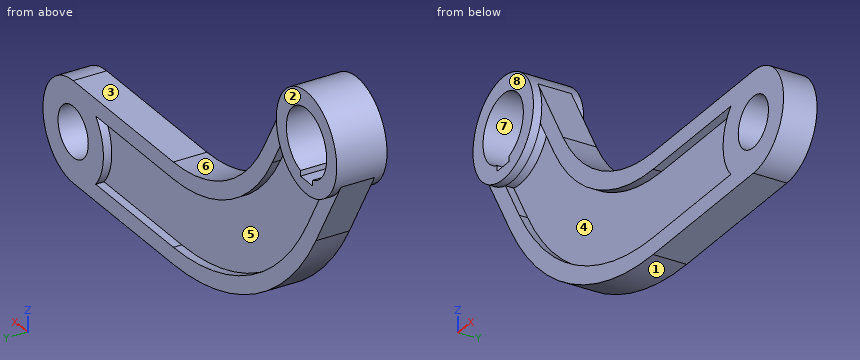
from build123d import *
from build123d.topology import SkipClean

# Parameters (mm, degrees)
SKETCH_1_R          = 30
EXTRUDE_1_DEPTH     = 15
SKETCH_2_R          = 15
EXTRUDE_2_DEPTH     = 10
SKETCH_3_R          = 30
SKETCH_3_R_2        = 15
EXTRUDE_3_DEPTH     = 10
CUT_EXTRUDE_1_DEPTH = 5
CUT_EXTRUDE_START   = -5
CUT_EXTRUDE_2_DEPTH = 5


with BuildPart() as part:
    # 草图1 → 凸台-拉伸1 (new, symmetric)
    with BuildSketch(Plane(origin=(0, 0, 0), x_dir=(1, 0, 0), z_dir=(0, 1, 0))):
        with Locations(Location((0, 0, 0), (0, 0, 270))):
            Circle(SKETCH_1_R)
        with BuildLine():
            Line((6, 19.078784028), (6, 22.378784028))
            Line((6, 22.378784028), (-6, 22.378784028))
            Line((-6, 22.378784028), (-6, 19.078784028))
            ThreePointArc((-6, 19.078784028), (0, -20), (6, 19.078784028))
        make_face(mode=Mode.SUBTRACT)
    extrude(amount=EXTRUDE_1_DEPTH, both=True)

    # 草图2 → 凸台-拉伸2 (add, symmetric)
    with BuildSketch(Plane(origin=(0, 0, 0), x_dir=(1, 0, 0), z_dir=(0, 1, 0))):
        with BuildLine():
            Line((-25.980762114, 15), (-0.980762114, 58.301270189))
            ThreePointArc((-0.980762114, 58.301270189), (58.826859022, 118.108891325), (140.525588833, 140))
            Line((140.525588833, 140), (240, 140))
            ThreePointArc((240, 140), (270, 110), (240, 80))
            Line((240, 80), (140.525588833, 80))
            ThreePointArc((140.525588833, 80), (88.826859022, 66.147367097), (50.980762114, 28.301270189))
            Line((50.980762114, 28.301270189), (25.980762114, -15))
            ThreePointArc((25.980762114, -15), (15, 25.980762114), (-25.980762114, 15))
        make_face()
        with Locations(Location((240, 110, 0), (0, 0, 270))):
            Circle(SKETCH_2_R, mode=Mode.SUBTRACT)
    extrude(amount=EXTRUDE_2_DEPTH, both=True)

    # 草图3 → 凸台-拉伸3 (add, symmetric)
    with BuildSketch(Plane(origin=(0, 0, 0), x_dir=(1, 0, 0), z_dir=(0, 1, 0))):
        with Locations((240, 110)):
            Circle(SKETCH_3_R)
        with Locations(Location((240, 110, 0), (0, 0, 270))):
            Circle(SKETCH_3_R_2, mode=Mode.SUBTRACT)
    extrude(amount=EXTRUDE_3_DEPTH, both=True)

    # 草图4 → 切除-拉伸1 (cut)
    with SkipClean():  # the faces are left unmerged after this step: merging them gives an invalid solid
        with BuildSketch(Plane(origin=(0, 10, 0), x_dir=(1, 0, 0), z_dir=(0, 1, 0))):
            with BuildLine():
                Line((217.639320225, 130), (140.525588833, 130))
                ThreePointArc((140.525588833, 130), (63.826859022, 109.448637287), (7.679491924, 53.301270189))
                Line((7.679491924, 53.301270189), (-6.140168188, 29.364916731))
                ThreePointArc((-6.140168188, 29.364916731), (15, 25.980762114), (28.500847963, 9.364916731))
                Line((28.500847963, 9.364916731), (42.320508076, 33.301270189))
                ThreePointArc((42.320508076, 33.301270189), (83.826859022, 74.807621135), (140.525588833, 90))
                Line((140.525588833, 90), (217.639320225, 90))
                ThreePointArc((217.639320225, 90), (210, 110), (217.639320225, 130))
            make_face()
        extrude(amount=-CUT_EXTRUDE_1_DEPTH, mode=Mode.SUBTRACT)

    # 草图5 → 切除-拉伸2 (cut)
    with SkipClean():  # the faces are left unmerged after this step: merging them gives an invalid solid
        with BuildSketch(Plane.XZ.offset(10).offset(CUT_EXTRUDE_START)):
            with BuildLine():
                Line((217.639320225, -90), (140.525588833, -90))
                ThreePointArc((140.525588833, -90), (83.826859022, -74.807621135), (42.320508076, -33.301270189))
                Line((42.320508076, -33.301270189), (28.500847963, -9.364916731))
                ThreePointArc((28.500847963, -9.364916731), (15, -25.980762114), (-6.140168188, -29.364916731))
                Line((-6.140168188, -29.364916731), (7.679491924, -53.301270189))
                ThreePointArc((7.679491924, -53.301270189), (63.826859022, -109.448637287), (140.525588833, -130))
                Line((140.525588833, -130), (217.639320225, -130))
                ThreePointArc((217.639320225, -130), (210, -110), (217.639320225, -90))
            make_face()
        extrude(amount=CUT_EXTRUDE_2_DEPTH, mode=Mode.SUBTRACT)


solid = part.part
Check sheet for the modelled part. Datum: model origin and axes. Units: mm. Face numbers are marked on the shaded views. A direction names the side the tool comes from. Round coordinates to 2 decimals unless told otherwise and drop trailing zeros. Loops run counter-clockwise (first coordinate to the right, second up) from the corner with the lowest first, then second, coordinate; pieces in that order, holes last.
1. Set-up check for the marked faces 1, 2, 3, 4 and 5: record each of +Z, -Z, +X, -X, +Y, -Y from which the full face is reachable in a straight line by a thin tool's end or side.
2. Sectioned sample at D-D on x = -10.5. Record the boundary of the cut face in (y, z).
3. Sectioned sample at A-A on y = -1. Record the boundary of the cut face in (x, z).
4. Sectioned sample at B-B on z = 0. Record the boundary of the cut face in (x, y).
5. Scan lines: probe 1 along X at (y, z) = (8.75, -13); probe 2 along Z at (x, y) = (0, -8.25); probe 3 along Y at (x, z) = (105, -75). Record each from-to range of solid material in increasing order.
6. Gauge pin test, flat ends, axial feed: pin 1 Ø10 at (y, z) = (-7, -51.5) entering from +X; pin 2 Ø1.5 at (x, y) = (196, 6.5) entering from +Z; pin 3 Ø2 at (y, z) = (0.5, -60.5) entering from -X; pin 4 Ø13 at (x, y) = (2.5, 6) entering from +Z. Record the tip position at first contact, or that the pin passes through.
7. Sectioned sample at C-C on x = 144.5. Record the boundary of the cut face in (y, z).
8. Mould release check, pull along X, two halves, no side actions. Record for the marked faces 6, 7 and 8: released by +X, released by -X, zero draft, split by the parting line, or undercut.
Recorded:
1. face 1: -Z, -X, +Y, -Y
1. face 2: +Z, -Z, +X, -X, +Y
1. face 3: +Z, +X, +Y, -Y
1. face 4: -Y
1. face 5: +Y
2. outline: (-15, -28.1) - (-10, -28.1) - (-10, -41.81) - (10, -41.81) - (10, -28.1) - (15, -28.1) - (15, -17.02) - (-15, -17.02) - close; (-15, 17.02) - (15, 17.02) - (15, 28.1) - (-15, 28.1) - close
3. outline: (-25.98, -15) - (-0.98, -58.3) arc R163.4 ccw to (140.53, -140) - (240, -140) arc R30 ccw to (240, -80) - (140.53, -80) arc R103.4 cw to (50.98, -28.3) - (25.98, 15) arc R30 ccw to start; hole (-6, -22.38) - (6, -22.38) - (6, -19.08) arc R20 ccw (long way) to (-6, -19.08) - close; hole circle Ø30 at (240, -110)
4. outline: (-30, -15) - (-20, -15) - (-20, 15) - (-30, 15) - close; (20, -15) - (30, -15) - (30, -10) - (34.64, -10) - (34.64, 10) - (30, 10) - (30, 15) - (20, 15) - close
5. probe 1: x = -27.04 to -15.2, 15.2 to 27.04, 30.6 to 42.15
5. probe 2: z = -59.98 to -40, -30 to -22.38, 20 to 30
5. probe 3: y = -10 to 10
6. pin 1: stops at x = 74.89
6. pin 2: stops at z = -80
6. pin 3: stops at x = -0.28
6. pin 4: stops at z = 30
7. outline: (-10, -140) - (10, -140) - (10, -130) - (5, -130) - (5, -90) - (10, -90) - (10, -80) - (-10, -80) - (-10, -90) - (-5, -90) - (-5, -130) - (-10, -130) - close
8. face 6: released by +X
8. face 7: undercut
8. face 8: zero draft
